For this review, take the finished solid that the model builds, in its own axes (mm). A direction names the side the tool comes from. Round coordinates to 2 decimals unless told otherwise and drop trailing zeros. Order: outer loops, then holes, each group sorted by start corner. A loop starts at its lowest first (then second) coordinate and runs counter-clockwise, first axis right, second up. Notation, with made-up numbers: (20, -8.75) -> (41, -8.75) arc R27 ccw to (41, 25.25) -> close; hole circle Ø1 at (31, 43). An arc over 180 degrees is marked (long way). Answer in a Markdown table with one row per item.
```python
from build123d import *

# Parameters (mm, degrees)
BASE_BLOCK_PROFILE_80X80_W  = 80
BASE_BLOCK_PROFILE_80X80_H  = 80
BASE_BLOCK_80X80X70_DEPTH   = 35
NOTCH_CUT_20X20_DEPTH       = 91
NOTCH_CUT_20X20_DEPTH_BACK  = 91
NOTCH_PROFILE_20X20_W       = 40
NOTCH_PROFILE_20X20_H       = 50
NOTCH_CUT_25X25_DEPTH       = 91
NOTCH_CUT_25X25_DEPTH_BACK  = 91
NOTCH_PROFILE_25X25_W       = 30
NOTCH_PROFILE_25X25_H       = 10
POCKET_CUT_40X15_DEPTH      = 97.046863561
POCKET_CUT_40X15_DEPTH_BACK = 97.046863561
POCKET_PROFILE_40X15_W      = 40
POCKET_PROFILE_40X15_H      = 10
UPRIGHT_SLOT_CUT_DEPTH      = 97.046863561
UPRIGHT_SLOT_CUT_DEPTH_BACK = 97.046863561
UPRIGHT_TOP_FILLETS_R20_R   = 20


with BuildPart() as part:
    # Base Block Profile 80x80 → Base Block 80x80x70 (new, symmetric)
    with BuildSketch(Plane(origin=(0, 0, 0), x_dir=(0, 0, -1), z_dir=(1, 0, 0))):
        Rectangle(BASE_BLOCK_PROFILE_80X80_W, BASE_BLOCK_PROFILE_80X80_H)
    extrude(amount=BASE_BLOCK_80X80X70_DEPTH, both=True)

    # Notch Profile 20x20 → Notch Cut 20x20 (cut, two sides: drawn at the far end of the back side and taken through both)
    with BuildSketch(Plane(origin=(35, 0, 0), x_dir=(0, 0, -1), z_dir=(1, 0, 0)).offset(-NOTCH_CUT_20X20_DEPTH_BACK)):
        with Locations((0, 15)):
            Rectangle(NOTCH_PROFILE_20X20_W, NOTCH_PROFILE_20X20_H)
    extrude(amount=NOTCH_CUT_20X20_DEPTH + NOTCH_CUT_20X20_DEPTH_BACK, mode=Mode.SUBTRACT)

    # Notch Profile 25x25 → Notch Cut 25x25 (cut, two sides: drawn at the far end of the back side and taken through both)
    with BuildSketch(Plane(origin=(35, 0, 0), x_dir=(0, 0, -1), z_dir=(1, 0, 0)).offset(-NOTCH_CUT_25X25_DEPTH_BACK)):
        with Locations((0, -35)):
            Rectangle(NOTCH_PROFILE_25X25_W, NOTCH_PROFILE_25X25_H)
    extrude(amount=NOTCH_CUT_25X25_DEPTH + NOTCH_CUT_25X25_DEPTH_BACK, mode=Mode.SUBTRACT)

    # Pocket Profile 40x15 → Pocket Cut 40x15 (cut, two sides: drawn at the far end of the back side and taken through both)
    with BuildSketch(Plane.XY.offset(40).offset(-POCKET_CUT_40X15_DEPTH_BACK)):
        with Locations((0, -35)):
            Rectangle(POCKET_PROFILE_40X15_W, POCKET_PROFILE_40X15_H)
    extrude(amount=POCKET_CUT_40X15_DEPTH + POCKET_CUT_40X15_DEPTH_BACK, mode=Mode.SUBTRACT)

    # Upright Slot Profile → Upright Slot Cut (cut, two sides: drawn at the far end of the back side and taken through both)
    with BuildSketch(Plane.XY.offset(40).offset(-UPRIGHT_SLOT_CUT_DEPTH_BACK)):
        with BuildLine():
            Line((-15, 26), (15, 26))
            ThreePointArc((15, 26), (23, 18), (15, 10))
            Line((15, 10), (-15, 10))
            ThreePointArc((-15, 10), (-23, 18), (-15, 26))
        make_face()
    extrude(amount=UPRIGHT_SLOT_CUT_DEPTH + UPRIGHT_SLOT_CUT_DEPTH_BACK, mode=Mode.SUBTRACT)

    # Upright Top Fillets R20
    upright_top_fillets_r20_edges = [part.edges().sort_by_distance(p)[0] for p in [
        (-35, 40, 30),
        (35, 40, 30),
        (-35, 40, -30),
        (35, 40, -30),
    ]]
    fillet(upright_top_fillets_r20_edges, radius=UPRIGHT_TOP_FILLETS_R20_R)


solid = part.part
```
Q1. Take a section at A-A, the plane x = -7. Write out the cut boundary in (y, z), then the cut area to 3 significant figures.
Answer key:
| item | result |
|---|---|
| outline | (-30, -40) -> (10, -40) -> (10, -20) -> (-10, -20) -> (-10, 20) -> (10, 20) -> (10, 40) -> (-30, 40) -> close; (26, -40) -> (40, -40) -> (40, -20) -> (26, -20) -> close; (26, 20) -> (40, 20) -> (40, 40) -> (26, 40) -> close |
| area | 2,960 mm^2 |
Q2. Take a section at B-B, the plane y = 3.5. Write out the cut boundary in (x, z).
Answer key:
| item | result |
|---|---|
| outline | (-35, -40) -> (35, -40) -> (35, -20) -> (-35, -20) -> close; (-35, 20) -> (35, 20) -> (35, 40) -> (-35, 40) -> close |
Q3. The part is to be moulded in two halves that separate along Y. For faces 1 (the face through (0, 10, -30)), 2 (the face through (0, -10, 0)), 3 (the face through (23, 18, -30)), 4 (the face through (28, -40, 28)), say which applies: +Y half, -Y half, draft (parallel to the pull), parting line (faces both ways), or undercut.
Answer key:
| item | result |
|---|---|
| face 1 | undercut |
| face 2 | +Y half |
| face 3 | undercut |
| face 4 | -Y half |
Q4. Clearance check with flat-ended pins moving along their axes: pin 1 Ø22 at (x, z) = (3, -27.5) entering from -Y; pin 2 Ø12 at (y, z) = (-32, 14) entering from +X. State where each tip first meets the part, or that it passes through.
Answer key:
| item | result |
|---|---|
| pin 1 | stops at y = -30 |
| pin 2 | stops at x = 35 |
Q5. Tool access review of faces 5 (the face through (-20, -35, 27)), 6 (the face through (29.297, 33.986, -30.14)), 7 (the face through (0, 9, 20)), 8 (the face through (-28, -35, 15)), 9 (the face through (23, 18, 30)): name each direction out of +Z, -Z, +X, -X, +Y, -Y from which nothing blocks a thin tool from reaching the whole face with its end or side.
Answer key:
| item | result |
|---|---|
| face 5 | +Z, -Z, -Y |
| face 6 | +Z, -Z, +X, +Y |
| face 7 | +X, -X, +Y |
| face 8 | +X, -X, -Y |
| face 9 | +Z, -Z |
Q6. Take a section at D-D, the plane z = 2. Write out the cut boundary in (x, y), then the cut area to 3 significant figures.
Answer key:
| item | result |
|---|---|
| outline | (-35, -30) -> (35, -30) -> (35, -10) -> (-35, -10) -> close |
| area | 1,400 mm^2 |
Q7. To check wall thickness, follow probe 1 along Y at (x, z) = (-1, 29.5); probe 2 along Z at (x, y) = (21, 32); probe 3 along Y at (x, z) = (-27.5, 13). State the ranges of each line that lie inside material, in increasing order.
Answer key:
| item | result |
|---|---|
| probe 1 | y = -30 to 10, 26 to 40 |
| probe 2 | z = -40 to -20, 20 to 40 |
| probe 3 | y = -30 to -10 |
Q8. Take a section at C-C, the plane y = 18. Write out the cut boundary in (x, z).
Answer key:
| item | result |
|---|---|
| outline | (-35, -40) -> (-23, -40) -> (-23, -20) -> (-35, -20) -> close; (-35, 20) -> (-23, 20) -> (-23, 40) -> (-35, 40) -> close; (23, -40) -> (35, -40) -> (35, -20) -> (23, -20) -> close; (23, 20) -> (35, 20) -> (35, 40) -> (23, 40) -> close |
